Source: CAD feature listing. Evaluate the final solid. Frame: model axes, mm. Face numbers are marked on the shaded views. A direction names the side the tool comes from. Coordinates: 2 decimals unless noted, no trailing zeros. Order: outer loops, then holes, each group sorted by start corner. A loop starts at its lowest first (then second) coordinate and runs counter-clockwise, first axis right, second up. Notation, with made-up numbers: (-19, 54.25) -> (40, 54.25) arc R25 ccw to (40, 71.25) -> close; hole circle Ø9 at (10.25, 29). An arc over 180 degrees is marked (long way). Put each result on its own line as item: value.
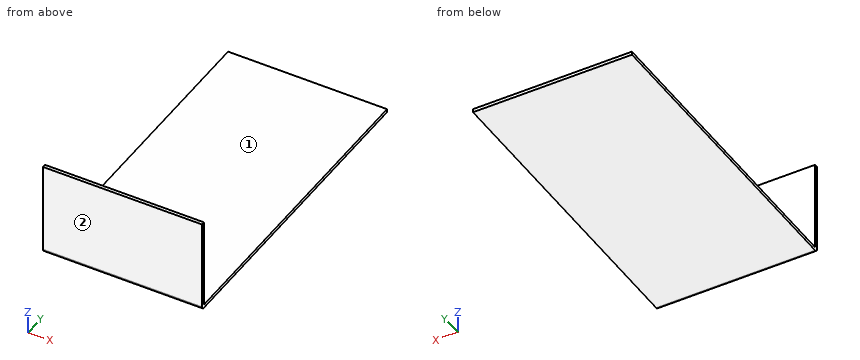
from build123d import *

# Parameters (mm, degrees)
SKETCH_1_W      = 140
SKETCH_1_H      = 280
EXTRUDE_1_DEPTH = 3
SKETCH_2_W      = 140
SKETCH_2_H      = 3
EXTRUDE_2_DEPTH = 80
FILLET_1_R      = 3


with BuildPart() as part:
    # 草图1 → 凸台-拉伸1 (new body)
    with BuildSketch(Plane.XY):
        with Locations((70, -140)):
            Rectangle(SKETCH_1_W, SKETCH_1_H)
    extrude(amount=EXTRUDE_1_DEPTH)

    # 草图2 → 凸台-拉伸2 (add)
    with BuildSketch(Plane.XY.offset(3)):
        with Locations((70, -278.5)):
            Rectangle(SKETCH_2_W, SKETCH_2_H)
    extrude(amount=EXTRUDE_2_DEPTH)

    # 圆角1
    fillet_1_edges = [part.edges().sort_by_distance(p)[0] for p in [
        (70, -280, 0),
    ]]
    fillet(fillet_1_edges, radius=FILLET_1_R)


solid = part.part
1. Cut plane C-C on y = -221.5. Output: boundary loops of the cut face in (x, z).
Numbers:
outline: (0, 0) -> (140, 0) -> (140, 3) -> (0, 3) -> close
2. Cut plane B-B on z = 48. Output: boundary loops of the cut face in (x, y), plus the area to 3 significant figures.
Numbers:
outline: (0, -280) -> (140, -280) -> (140, -277) -> (0, -277) -> close
area: 420 mm2
3. Cut plane A-A on x = 26. Output: boundary loops of the cut face in (y, z), plus the area to 3 significant figures.
Numbers:
outline: (-280, 3) arc R3 ccw to (-277, 0) -> (0, 0) -> (0, 3) -> (-277, 3) -> (-277, 83) -> (-280, 83) -> close
area: 1,080 mm2
4. First-contact query: pin 1 (4 mm diameter, centred on x = 30, y = -182, fed in from +Z); pin 2 (2 mm diameter, centred on x = 60, z = 67, fed in from +Y). Flat tips, straight axial feed; report the tip coordinate or a pass-through.
Numbers:
pin 1: stops at z = 3
pin 2: stops at y = -277
5. Ray query, line 1 along Z through (x, y) = (108.5, -15.5); line 2 along Y through (x, z) = (9, 61). Return the intervals inside material, ascending.
Numbers:
line 1: z = 0 to 3
line 2: y = -280 to -277
6. Set-up query: the marked faces 1 and 2. Return all of +Z, -Z, +X, -X, +Y, -Y with unobstructed straight access to the full face (end or side cutting, diameter ignored); none if empty.
Numbers:
face 1: +Z, +X, -X, +Y
face 2: +Z, -Z, +X, -X, -Y
